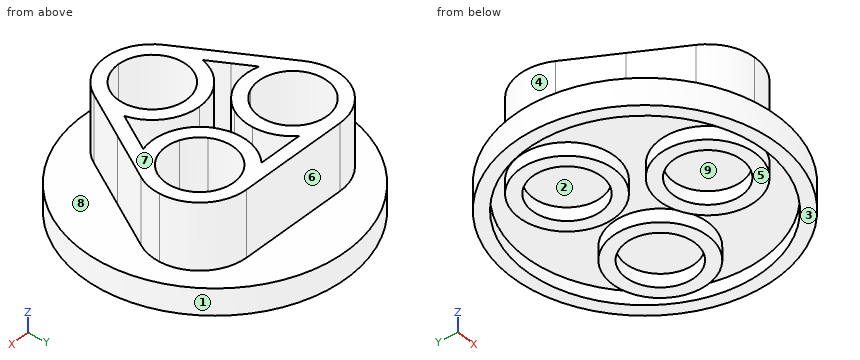
from build123d import *

# Parameters (mm, degrees)
FLANGE_PROFILE_100_R       = 50
FLANGE_100X10_DEPTH        = 10
TUBE_CLUSTER_BOSS_DEPTH    = 25
FLANGE_RECESS_PROFILE_90_R = 45
FLANGE_RECESS_90X5_DEPTH   = 5
HOLLOW_START               = -35
TUBE_PROFILES_3X_36_26_R   = 18
TUBE_PROFILES_3X_36_26_R_2 = 13
HOLLOW_TUBES_3X_36_DEPTH   = 35


with BuildPart() as part:
    # Flange Profile _100 → Flange _100x10 (new body)
    with BuildSketch(Plane.XY):
        Circle(FLANGE_PROFILE_100_R)
    extrude(amount=FLANGE_100X10_DEPTH)

    # Tube Cluster Boss Profile → Tube Cluster Boss (add)
    with BuildSketch(Plane.XY.offset(10)):
        with BuildLine():
            ThreePointArc((-8.334710093, 25), (-14.076405758, 28.703293088), (-20.784609691, 30))
            ThreePointArc((-20.784609691, 30), (-36.373066959, 21), (-36.373066959, 3))
            ThreePointArc((-36.373066959, 3), (-31.895983866, -2.161121564), (-25.817990141, -5.281929326))
            ThreePointArc((-25.817990141, -5.281929326), (-15.830471874, -5.304812004), (-7.368201826, 0))
            Line((-7.368201826, 0), (-15.784609691, 0))
            ThreePointArc((-15.784609691, 0), (-31.601263517, 19.211102551), (-7.784609691, 12))
            ThreePointArc((-7.784609691, 12), (-8.227573949, 8.635352414), (-9.526279442, 5.5))
            Line((-9.526279442, 5.5), (-5.196152423, 3))
            ThreePointArc((-5.196152423, 3), (-3.397944818, 7.341257188), (-2.784609691, 12))
            ThreePointArc((-2.784609691, 12), (-4.23018139, 19.067595321), (-8.334710093, 25))
        make_face()
        with BuildLine():
            Line((-15.784609691, 0), (-7.368201826, 0))
            ThreePointArc((-7.368201826, 0), (-6.204810298, 1.443985143), (-5.196152423, 3))
            Line((-5.196152423, 3), (-9.526279442, 5.5))
            ThreePointArc((-9.526279442, 5.5), (-12.202895082, 2.235053795), (-15.784609691, 0))
        make_face()
        with BuildLine():
            ThreePointArc((-25.817990141, -5.281929326), (-31.895983866, -2.161121564), (-36.373066959, 3))
            Line((-36.373066959, 3), (-25.980762114, -15))
            Line((-25.980762114, -15), (-21.650635095, -12.5))
            Line((-21.650635095, -12.5), (-25.817990141, -5.281929326))
        make_face()
        with BuildLine():
            Line((-21.650635095, -12.5), (-25.980762114, -15))
            Line((-25.980762114, -15), (-15.588457268, -33))
            ThreePointArc((-15.588457268, -33), (-17.819578108, -26.542171525), (-17.483280048, -19.718070674))
            Line((-17.483280048, -19.718070674), (-21.650635095, -12.5))
        make_face()
        with BuildLine():
            ThreePointArc((17.483280048, -19.718070674), (11.111374175, -9.838878436), (0, -6))
            Line((0, -6), (0, -11))
            ThreePointArc((0, -11), (9.192388155, -14.807611845), (13, -24))
            ThreePointArc((13, -24), (9.192388155, -33.192388155), (0, -37))
            Line((0, -37), (0, -42))
            ThreePointArc((0, -42), (9, -39.588457268), (15.588457268, -33))
            ThreePointArc((15.588457268, -33), (17.386664873, -28.658742812), (18, -24))
            ThreePointArc((18, -24), (17.870353114, -21.843502941), (17.483280048, -19.718070674))
        make_face()
        with BuildLine():
            Line((0, -11), (0, -6))
            ThreePointArc((0, -6), (-11.111374175, -9.838878436), (-17.483280048, -19.718070674))
            ThreePointArc((-17.483280048, -19.718070674), (-17.819578108, -26.542171525), (-15.588457268, -33))
            ThreePointArc((-15.588457268, -33), (-9, -39.588457268), (0, -42))
            Line((0, -42), (0, -37))
            ThreePointArc((0, -37), (-13, -24), (0, -11))
        make_face()
        with BuildLine():
            Line((21.650635095, -12.5), (17.483280048, -19.718070674))
            ThreePointArc((17.483280048, -19.718070674), (17.870353114, -21.843502941), (18, -24))
            ThreePointArc((18, -24), (17.386664873, -28.658742812), (15.588457268, -33))
            Line((15.588457268, -33), (25.980762114, -15))
            Line((25.980762114, -15), (21.650635095, -12.5))
        make_face()
        with BuildLine():
            Line((25.980762114, -15), (36.373066959, 3))
            ThreePointArc((36.373066959, 3), (31.895983866, -2.161121564), (25.817990141, -5.281929326))
            Line((25.817990141, -5.281929326), (21.650635095, -12.5))
            Line((21.650635095, -12.5), (25.980762114, -15))
        make_face()
        with BuildLine():
            ThreePointArc((38.784609691, 12), (33.512531752, 24.727922061), (20.784609691, 30))
            ThreePointArc((20.784609691, 30), (14.076405758, 28.703293088), (8.334710093, 25))
            ThreePointArc((8.334710093, 25), (2.965031583, 14.542171525), (5.196152423, 3))
            Line((5.196152423, 3), (9.526279442, 5.5))
            ThreePointArc((9.526279442, 5.5), (17.419962104, 24.557035742), (33.784609691, 12))
            ThreePointArc((33.784609691, 12), (27.995712242, 1.183346174), (15.784609691, 0))
            Line((15.784609691, 0), (7.368201826, 0))
            ThreePointArc((7.368201826, 0), (15.830471874, -5.304812004), (25.817990141, -5.281929326))
            ThreePointArc((25.817990141, -5.281929326), (31.895983866, -2.161121564), (36.373066959, 3))
            ThreePointArc((36.373066959, 3), (38.171274564, 7.341257188), (38.784609691, 12))
        make_face()
        with BuildLine():
            Line((9.526279442, 5.5), (5.196152423, 3))
            ThreePointArc((5.196152423, 3), (6.204810298, 1.443985143), (7.368201826, 0))
            Line((7.368201826, 0), (15.784609691, 0))
            ThreePointArc((15.784609691, 0), (12.202895082, 2.235053795), (9.526279442, 5.5))
        make_face()
        with BuildLine():
            Line((20.784609691, 30), (0, 30))
            Line((0, 30), (0, 25))
            Line((0, 25), (8.334710093, 25))
            ThreePointArc((8.334710093, 25), (14.076405758, 28.703293088), (20.784609691, 30))
        make_face()
        with BuildLine():
            Line((0, 25), (0, 30))
            Line((0, 30), (-20.784609691, 30))
            ThreePointArc((-20.784609691, 30), (-14.076405758, 28.703293088), (-8.334710093, 25))
            Line((-8.334710093, 25), (0, 25))
        make_face()
    extrude(amount=TUBE_CLUSTER_BOSS_DEPTH)

    # Flange Recess Profile _90 → Flange Recess _90x5 (cut)
    with BuildSketch(Plane(origin=(0, 0, 0), x_dir=(-1, 0, 0), z_dir=(0, 0, -1))):
        Circle(FLANGE_RECESS_PROFILE_90_R)
    extrude(amount=-FLANGE_RECESS_90X5_DEPTH, mode=Mode.SUBTRACT)

    # Tube Profiles 3x_36-_26 → Hollow Tubes 3x_36 (add)
    # profile 1 of 3: a face of its own
    with BuildSketch(Plane.XY.offset(35).offset(HOLLOW_START)):
        with Locations((20.784609691, 12)):
            Circle(TUBE_PROFILES_3X_36_26_R)
        with Locations((20.784609691, 12)):
            Circle(TUBE_PROFILES_3X_36_26_R_2, mode=Mode.SUBTRACT)
    # profile 2 of 3: a face of its own
    with BuildSketch(Plane.XY.offset(35).offset(HOLLOW_START)):
        with Locations((-20.784609691, 12)):
            Circle(TUBE_PROFILES_3X_36_26_R)
        with Locations((-20.784609691, 12)):
            Circle(TUBE_PROFILES_3X_36_26_R_2, mode=Mode.SUBTRACT)
    # profile 3 of 3: a face of its own
    with BuildSketch(Plane.XY.offset(35).offset(HOLLOW_START)):
        with Locations((0, -24)):
            Circle(TUBE_PROFILES_3X_36_26_R)
        with Locations((0, -24)):
            Circle(TUBE_PROFILES_3X_36_26_R_2, mode=Mode.SUBTRACT)
    extrude(amount=HOLLOW_TUBES_3X_36_DEPTH)


solid = part.part
Verification items for the finished model (mm, model axes). Face numbers are marked on the shaded views. A direction names the side the tool comes from. Coordinates: 2 decimals unless noted, no trailing zeros. Order: outer loops, then holes, each group sorted by start corner. A loop starts at its lowest first (then second) coordinate and runs counter-clockwise, first axis right, second up. Notation, with made-up numbers: (67.5, -13.5) -> (75.5, -13.5) arc R24 ccw to (75.5, 13.5) -> close; hole circle Ø9 at (-15, -40). An arc over 180 degrees is marked (long way). Put each result on its own line as item: value. Start each with the question number.
1. Mould release check, pull along X, two halves, no side actions. Record for the marked faces 1, 2, 3 and 4: released by +X, released by -X, zero draft, split by the parting line, or undercut.
2. Cross-section at A-A, the plane z = 3. Record the boundary of the cut face in (x, y), then the cut area to 3 significant figures.
3. Cross-section at C-C, the plane x = 42.5. Record the boundary of the cut face in (y, z).
4. Access from +Z, -Z, +X, -X, +Y, -Y to the whole of each face (thin tool, end or side, straight path). Record for the marked faces 5, 6, 7, 8 and 9.
5. Cross-section at D-D, the plane x = 32.5. Record the boundary of the cut face in (y, z).
6. Go/stop test with flat-tipped pins: pin 1 Ø21 at (x, y) = (0, -24) entering from -Z; pin 2 Ø8 at (x, y) = (22.5, 15.5) entering from +Z; pin 3 Ø1 at (y, z) = (-12.5, 17) entering from -X. Record where each tip stops, or that it passes through.
7. Cross-section at B-B, the plane z = 32. Record the boundary of the cut face in (x, y).
8. Material ranges on L1, parallel to X at y = 6, z = 28; L2, parallel to Y at x = 0, z = 2.8; L3, parallel to X at y = 12, z = 3.15, recorded low to high. Write a range as [from, to].
Computed:
1. face 1: split by the parting line
1. face 2: undercut
1. face 3: zero draft
1. face 4: released by -X
2. outline: circle Ø100 at (0, 0); circle Ø36 at (-20.78, 12); circle Ø36 at (0, -24); circle Ø36 at (20.78, 12); hole circle Ø90 at (0, 0); hole circle Ø26 at (-20.78, 12); hole circle Ø26 at (0, -24); hole circle Ø26 at (20.78, 12)
2. area: 2,950 mm2
3. outline: (-26.34, 0) -> (-14.79, 0) -> (-14.79, 5) -> (14.79, 5) -> (14.79, 0) -> (26.34, 0) -> (26.34, 10) -> (-26.34, 10) -> close
4. face 5: -Z, +X, -X, +Y, -Y
4. face 6: +Z, +X, -X, +Y
4. face 7: +Z, +X, -X, +Y, -Y
4. face 8: +Z
4. face 9: -Z
5. outline: (-38, 0) -> (-31.12, 0) -> (-31.12, 5) -> (-1.67, 5) -> (-1.67, 0) -> (6.37, 0) -> (6.37, 5) -> (17.63, 5) -> (17.63, 0) -> (25.67, 0) -> (25.67, 5) -> (31.12, 5) -> (31.12, 0) -> (38, 0) -> (38, 10) -> (25.67, 10) -> (25.67, 35) -> (17.63, 35) -> (17.63, 10) -> (6.37, 10) -> (6.37, 35) -> (-3.71, 35) -> (-3.71, 10) -> (-38, 10) -> close
6. pin 1: z = 5
6. pin 2: z = 10
6. pin 3: x = -27.71
7. outline: (-36.37, 3) -> (-15.59, -33) arc R18 ccw to (15.59, -33) -> (36.37, 3) arc R18 ccw to (20.78, 30) -> (-20.78, 30) arc R18 ccw to start; hole circle Ø26 at (-20.78, 12); hole (-25.82, -5.28) -> (-17.48, -19.72) arc R18 cw to (17.48, -19.72) -> (25.82, -5.28) arc R18 cw to (8.33, 25) -> (-8.33, 25) arc R18 cw to start; hole circle Ø26 at (0, -24); hole circle Ø26 at (20.78, 12)
8. L1: [-37.76, -32.32], [-9.25, -3.81], [3.81, 9.25], [32.32, 37.76]
8. L2: [-50, -45], [-42, -37], [-11, -6], [45, 50]
8. L3: [-48.54, -43.37], [-38.78, -33.78], [-7.78, -2.78], [2.78, 7.78], [33.78, 38.78], [43.37, 48.54]
